Verification items for the finished model (mm, model axes). Round coordinates to 2 decimals unless told otherwise and drop trailing zeros. Write each loop counter-clockwise with the first axis right and the second up, starting at its lowest first coordinate (ties: lowest second). Pieces come first, ordered by that corner, then holes. Notation, with made-up numbers: (40.5, -23.75) - (63.5, -23.75) arc R38 ccw to (63.5, 15.25) - close; hole circle Ø8 at (3.25, 38). An arc over 180 degrees is marked (long way). Answer as a JSON object with one key per item and string values.
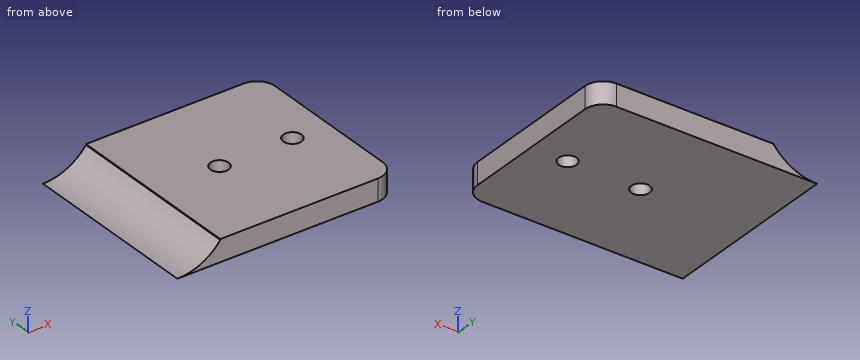
```python
from build123d import *

# Parameters (mm, degrees)
BOSS_EXTRUDE1_DEPTH   = 6
BOSS_EXTRUDE2_DEPTH   = 50
M6_TAPPED_HOLE1_D     = 5
M6_TAPPED_HOLE1_DEPTH = 15
M6_TAPPED_HOLE1_TIP   = 1.502151548


with BuildPart() as part:
    # Sketch1 → Boss-Extrude1 (new body)
    with BuildSketch(Plane.XY.offset(-15)):
        with BuildLine():
            Line((11.8, -5), (55, -5))
            ThreePointArc((55, -5), (58.535533906, -6.464466094), (60, -10))
            Line((60, -10), (60, -50))
            ThreePointArc((60, -50), (58.535533906, -53.535533906), (55, -55))
            Line((55, -55), (11.8, -55))
            Line((11.8, -55), (11.8, -5))
        make_face()
    extrude(amount=BOSS_EXTRUDE1_DEPTH)

    # Sketch2 → Boss-Extrude2 (add)
    with BuildSketch(Plane(origin=(0, -5, 0), x_dir=(1, 0, 0), z_dir=(0, 1, 0))):
        with BuildLine():
            Line((0, 15), (11.8, 15))
            Line((11.8, 15), (11.8, 9.260669522))
            ThreePointArc((11.8, 9.260669522), (6.560867213, 13.489070443), (0, 15))
        make_face()
    extrude(amount=-BOSS_EXTRUDE2_DEPTH)

    # M6 Tapped Hole1
    with Locations(Plane(origin=(50, -30, -9), x_dir=(1, 0, 0), z_dir=(0, 0, 1))):
        with Locations((0, 0), (-20, 0)):
            Hole(M6_TAPPED_HOLE1_D / 2, depth=M6_TAPPED_HOLE1_DEPTH)
            with Locations((0, 0, -(M6_TAPPED_HOLE1_DEPTH + M6_TAPPED_HOLE1_TIP / 2))):  # 118° drill point
                Cone(0, M6_TAPPED_HOLE1_D / 2, M6_TAPPED_HOLE1_TIP, mode=Mode.SUBTRACT)


solid = part.part
```
1. Cross-section at D-D (y = -16). Record the boundary of the cut face in (x, z).
Completed:
{"outline": "(0, -15) - (60, -15) - (60, -9) - (11.8, -9) - (11.8, -9.26) arc R15 cw to start"}
2. Cross-section at B-B (y = -30). Record the boundary of the cut face in (x, z).
Completed:
{"outline": "(0, -15) - (27.5, -15) - (27.5, -9) - (11.8, -9) - (11.8, -9.26) arc R15 cw to start; (32.5, -15) - (47.5, -15) - (47.5, -9) - (32.5, -9) - close; (52.5, -15) - (60, -15) - (60, -9) - (52.5, -9) - close"}
3. Material ranges on probe 1 along Y at (x, z) = (50, -12.5); probe 2 along Y at (x, z) = (50.5, -11.85); probe 3 along X at (y, z) = (-22, -10.05), recorded low to high. Write a range as from..to.
Completed:
{"probe 1": "y = -55..-32.5, -27.5..-5", "probe 2": "y = -55..-32.45, -27.55..-5", "probe 3": "x = 11.14..60"}
4. Cross-section at C-C (z = -14.05). Record the boundary of the cut face in (x, y), plus the area to 3 significant figures.
Completed:
{"outline": "(5.25, -55) - (55, -55) arc R5 ccw to (60, -50) - (60, -10) arc R5 ccw to (55, -5) - (5.25, -5) - close; hole circle Ø5 at (30, -30); hole circle Ø5 at (50, -30)", "area": "2,690 mm^2"}
5. Cross-section at A-A (x = 50). Record the boundary of the cut face in (y, z).
Completed:
{"outline": "(-55, -15) - (-32.5, -15) - (-32.5, -9) - (-55, -9) - close; (-27.5, -15) - (-5, -15) - (-5, -9) - (-27.5, -9) - close"}
